from build123d import *

# Parameters (mm, degrees)
RIM_LIP_SKETCH_210_R      = 105
RIM_LIP_210_DEPTH         = 5
FRONT_FLANGE_SKETCH_200_R = 100
FRONT_FLANGE_200_DEPTH    = 38
HUB_BARREL_SKETCH_100_R   = 50
HUB_BARREL_100_DEPTH      = 62
REAR_FLANGE_SKETCH_200_R  = 100
REAR_FLANGE_200_DEPTH     = 22
FRONT_RECESS_SKETCH_185_R = 92.5
FRONT_RECESS_185_DEPTH    = 23
BORE_SKETCH_60_R          = 30
BORE_60_DEPTH             = 182.289823211
FLANGE_HOLES_SKETCH_R     = 11
FLANGE_HOLES_SKETCH_R_2   = 8.25
FLANGE_HOLES_DEPTH        = 182.289823211


with BuildPart() as part:
    # Rim Lip Sketch Ø210 → Rim Lip Ø210 (new body)
    with BuildSketch(Plane.XY):
        Circle(RIM_LIP_SKETCH_210_R)
    extrude(amount=-RIM_LIP_210_DEPTH)

    # Front Flange Sketch Ø200 → Front Flange Ø200 (add)
    with BuildSketch(Plane(origin=(0, 0, -5), x_dir=(-1, 0, 0), z_dir=(0, 0, -1))):
        Circle(FRONT_FLANGE_SKETCH_200_R)
    extrude(amount=FRONT_FLANGE_200_DEPTH)

    # Hub Barrel Sketch Ø100 → Hub Barrel Ø100 (add)
    with BuildSketch(Plane(origin=(0, 0, -43), x_dir=(-1, 0, 0), z_dir=(0, 0, -1))):
        Circle(HUB_BARREL_SKETCH_100_R)
    extrude(amount=HUB_BARREL_100_DEPTH)

    # Rear Flange Sketch Ø200 → Rear Flange Ø200 (add)
    with BuildSketch(Plane(origin=(0, 0, -105), x_dir=(-1, 0, 0), z_dir=(0, 0, -1))):
        Circle(REAR_FLANGE_SKETCH_200_R)
    extrude(amount=REAR_FLANGE_200_DEPTH)

    # Front Recess Sketch Ø185 → Front Recess Ø185 (cut)
    with BuildSketch(Plane.XY):
        Circle(FRONT_RECESS_SKETCH_185_R)
    extrude(amount=-FRONT_RECESS_185_DEPTH, mode=Mode.SUBTRACT)

    # Bore Sketch Ø60 → Bore Ø60 (cut, through all)
    with BuildSketch(Plane.XY.offset(-23)):
        Circle(BORE_SKETCH_60_R)
    extrude(amount=-BORE_60_DEPTH, mode=Mode.SUBTRACT)

    # Flange Holes Sketch → Flange Holes (cut, through all)
    with BuildSketch(Plane.XY.offset(-23)):
        with Locations((0, 75)):
            Circle(FLANGE_HOLES_SKETCH_R)
        with Locations((64.951905284, 37.5)):
            Circle(FLANGE_HOLES_SKETCH_R)
        with Locations((64.951905284, -37.5)):
            Circle(FLANGE_HOLES_SKETCH_R)
        with Locations((0, -75)):
            Circle(FLANGE_HOLES_SKETCH_R)
        with Locations((-64.951905284, -37.5)):
            Circle(FLANGE_HOLES_SKETCH_R)
        with Locations((-64.951905284, 37.5)):
            Circle(FLANGE_HOLES_SKETCH_R)
        with Locations((-71.25, 0)):
            Circle(FLANGE_HOLES_SKETCH_R_2)
        with Locations((71.25, 0)):
            Circle(FLANGE_HOLES_SKETCH_R_2)
        with Locations((35.625, -61.70431002)):
            Circle(FLANGE_HOLES_SKETCH_R_2)
        with Locations((-35.625, 61.70431002)):
            Circle(FLANGE_HOLES_SKETCH_R_2)
    extrude(amount=-FLANGE_HOLES_DEPTH, mode=Mode.SUBTRACT)


solid = part.part
Can you work these out from the model? Positions are in its coordinate system, mm. A direction names the side the tool comes from. Coordinates: 2 decimals unless noted, no trailing zeros. Loops run counter-clockwise (first coordinate to the right, second up) from the corner with the lowest first, then second, coordinate; pieces in that order, holes last. Notation, with made-up numbers: (66, -35.5) - (117, -35.5) arc R9 cw to (117, -20.5) - close; hole circle Ø11 at (52, 23.25). An arc over 180 degrees is marked (long way). Answer as a JSON object with one key per item and string values. Group by question number.
Item 1: On a 3-axis mill with a long thin cutter (end or side, diameter ignored), from which of +Z, -Z, +X, -X, +Y, -Y can I reach the whole of each face in a straight line? I mean faces 1 (the face through (93, -38, -5)), 2 (the face through (49.727, 77.996, -11.339)), 3 (the face through (-54.46, 40.8, -32.86)). Say none if no direction works.
Item 2: If we mould it in two halves opening along X, with no side actions, what happens to faces 4 (the face through (-95.38, 30.04, -115.85)), 5 (the face through (46, -21, -43)), 6 (the face through (33.84, -69.76, -115.85))? For each: released by +X, released by -X, zero draft, split by the parting line, or undercut.
Item 3: For pin 1 (20 mm diameter, centred on x = 0, y = 75, fed in from -Z); pin 2 (10 mm diameter, centred on x = -17.5, y = -78.5, fed in from +Z); pin 3 (2 mm diameter, centred on x = 30, z = -86.5, fed in from -Y); pin 4 (12 mm diameter, centred on y = 82, z = -34.5, fed in from -X), each with a flat end and sliding along its axis, tell me the tip position at first contact or that it passes through.
Item 4: If we section it at B-B (z = -69): List the corners of the cut face in (x, y) for me.
Item 5: If we section it at A-A (y = 75): List the corners of the cut face in (x, z) for me, plus the area to 3 significant figures.
Item 6: If we section it at D-D (y = 23): List the corners of the cut face in (x, z) for me.
Item 7: If we section it at C-C (x = 0): State how many separate pieces and enclosed holes the cut face has, plus the area to 3 significant figures.
Item 8: If I drill on L1, parallel to Z at x = 59, y = -12; L2, parallel to Y at x = 59.5, z = -26; L3, parallel to Z at x = 39, y = 84, over which ranges is the centre line in solid material (lowest first)? Write a range as from..to.
Returned:
{
 "1": {"face 1": "-Z", "face 2": "+Z", "face 3": "+Z, -Z"},
 "2": {"face 4": "split by the parting line", "face 5": "zero draft", "face 6": "undercut"},
 "3": {"pin 1": "passes through", "pin 2": "stops at z = -23", "pin 3": "stops at y = -40.73", "pin 4": "stops at x = -64.99"},
 "4": {"outline": "circle Ø100 at (0, 0); hole circle Ø60 at (0, 0)"},
 "5": {"outline": "(-73.48, -5) - (-66.14, -5) - (-66.14, -43) - (-11, -43) - (-11, -23) - (-54.14, -23) - (-54.14, 0) - (-73.48, 0) - close; (-66.14, -127) - (-11, -127) - (-11, -105) - (-66.14, -105) - close; (11, -127) - (66.14, -127) - (66.14, -105) - (11, -105) - close; (11, -43) - (66.14, -43) - (66.14, -5) - (73.48, -5) - (73.48, 0) - (54.14, 0) - (54.14, -23) - (11, -23) - close", "area": "5,260 mm²"},
 "6": {"outline": "(-102.45, -5) - (-97.32, -5) - (-97.32, -43) - (-44.4, -43) - (-44.4, -105) - (-97.32, -105) - (-97.32, -127) - (-19.26, -127) - (-19.26, -23) - (-89.59, -23) - (-89.59, 0) - (-102.45, 0) - close; (19.26, -127) - (97.32, -127) - (97.32, -105) - (44.4, -105) - (44.4, -43) - (97.32, -43) - (97.32, -5) - (102.45, -5) - (102.45, 0) - (89.59, 0) - (89.59, -23) - (19.26, -23) - close"},
 "7": {"separate pieces": "6", "enclosed holes": "0", "area": "6,910 mm²"},
 "8": {"L1": "z = -127..-105, -43..-23", "L2": "y = -80.37..-47.05, -27.95..27.95, 47.05..80.37", "L3": "z = -127..-105, -43..0"}
}
